```python
from build123d import *

# Parameters (mm, degrees)
BOSS_EXTRUDE1_DEPTH = 1681


with BuildPart() as part:
    # Sketch1 → Boss-Extrude1 (new body)
    with BuildSketch(Plane.XY):
        with BuildLine():
            Line((0, 0), (250, 0))
            Line((250, 0), (250, 14))
            Line((250, 14), (142.5, 14))
            ThreePointArc((142.5, 14), (133.307611845, 17.807611845), (129.5, 27))
            Line((129.5, 27), (129.5, 223))
            ThreePointArc((129.5, 223), (133.307611845, 232.192388155), (142.5, 236))
            Line((142.5, 236), (250, 236))
            Line((250, 236), (250, 250))
            Line((250, 250), (0, 250))
            Line((0, 250), (0, 236))
            Line((0, 236), (107.5, 236))
            ThreePointArc((107.5, 236), (116.692388155, 232.192388155), (120.5, 223))
            Line((120.5, 223), (120.5, 27))
            ThreePointArc((120.5, 27), (116.692388155, 17.807611845), (107.5, 14))
            Line((107.5, 14), (0, 14))
            Line((0, 14), (0, 0))
        make_face()
    extrude(amount=BOSS_EXTRUDE1_DEPTH)


solid = part.part
```
Geometry: final body of the model. Coordinates: model frame, mm. A direction names the side the tool comes from. Coordinates: 2 decimals unless noted, no trailing zeros. Order: outer loops, then holes, each group sorted by start corner. A loop starts at its lowest first (then second) coordinate and runs counter-clockwise, first axis right, second up. Notation, with made-up numbers: (27, 72) -> (82, 72) arc R6 cw to (82, 76) -> close; hole circle Ø10 at (-18.75, 29). An arc over 180 degrees is marked (long way). Answer in a Markdown table with one row per item.
Item 1: Section C-C on y = 152.5. Output: boundary loops of the cut face in (x, z), plus the area to 3 significant figures.
Return value:
| item | result |
|---|---|
| outline | (120.5, 0) -> (129.5, 0) -> (129.5, 1681) -> (120.5, 1681) -> close |
| area | 15,100 mm² |
Item 2: Ray query, L1, parallel to Y at x = 55, z = 668; L2, parallel to X at y = 158, z = 371.5; L3, parallel to Y at x = 111, z = 1079.5. Return the intervals inside material, ascending.
Return value:
| item | result |
|---|---|
| L1 | y = 0 to 14, 236 to 250 |
| L2 | x = 120.5 to 129.5 |
| L3 | y = 0 to 14.48, 235.52 to 250 |
Item 3: Access query for faces 4 (the flat face through (124, 163, 0)), 5 (the flat face through (53, 236, 829)), 6 (the flat face through (129.5, 124, 829)). Directions: +Z, -Z, +X, -X, +Y, -Y. A direction counts if a zero-diameter tool reaches every point of the face in a straight line with its end or side. Return the directions, or none.
Return value:
| item | result |
|---|---|
| face 4 | -Z, +X, -X, +Y, -Y |
| face 5 | +Z, -Z, -X |
| face 6 | +Z, -Z, +X |
Item 4: Section B-B on z = 205. Output: boundary loops of the cut face in (x, y), plus the area to 3 significant figures.
Return value:
| item | result |
|---|---|
| outline | (0, 0) -> (250, 0) -> (250, 14) -> (142.5, 14) arc R13 cw to (129.5, 27) -> (129.5, 223) arc R13 cw to (142.5, 236) -> (250, 236) -> (250, 250) -> (0, 250) -> (0, 236) -> (107.5, 236) arc R13 cw to (120.5, 223) -> (120.5, 27) arc R13 cw to (107.5, 14) -> (0, 14) -> close |
| area | 9,140 mm² |
Item 5: Contact query for flat-ended pins moving along their axis: P1, Ø12, axis at y = 162, z = 170.5, coming from the +X side; P2, Ø5, axis at y = 60.5, z = 1173, coming from the -X side. Output: stop coordinate, or through.
Return value:
| item | result |
|---|---|
| P1 | stops at x = 129.5 |
| P2 | stops at x = 120.5 |
Item 6: Section A-A on x = 44.5. Output: boundary loops of the cut face in (y, z).
Return value:
| item | result |
|---|---|
| outline | (0, 0) -> (14, 0) -> (14, 1681) -> (0, 1681) -> close; (236, 0) -> (250, 0) -> (250, 1681) -> (236, 1681) -> close |
Item 7: Draft query along Y for faces 1 (the flat face through (124, 163, 1681)), 2 (the flat face through (127, 250, 829)), 3 (the flat face through (195, 236, 829)). Return one class per face: released by +Y, released by -Y, zero draft, split by the parting line, or undercut.
Return value:
| item | result |
|---|---|
| face 1 | zero draft |
| face 2 | released by +Y |
| face 3 | undercut |
